Geometry: final body of the model. Coordinates: model frame, mm. A direction names the side the tool comes from. Give positions to 0.01 mm unless a question says otherwise; leave off trailing zeros. Order: outer loops, then holes, each group sorted by start corner. A loop starts at its lowest first (then second) coordinate and runs counter-clockwise, first axis right, second up. Notation, with made-up numbers: (44.5, -37) -> (78.5, -37) arc R34 cw to (78.5, 2) -> close; hole circle Ø11 at (17.25, -7). An arc over 180 degrees is marked (long way). Write item = value, one per line.
```python
from build123d import *

# Parameters (mm, degrees)
BOSS_EXTRUDE1_DEPTH = 12.7


with BuildPart() as part:
    # Sketch1 → Boss-Extrude1 (new, symmetric)
    with BuildSketch(Plane.XY):
        with BuildLine():
            Line((0, 79.375), (19.05, 79.375))
            Line((19.05, 79.375), (19.05, 69.375))
            Line((19.05, 69.375), (0, 69.375))
            ThreePointArc((0, 69.375), (-69.375, 0), (0, -69.375))
            Line((0, -69.375), (19.05, -69.375))
            Line((19.05, -69.375), (19.05, -79.375))
            Line((19.05, -79.375), (0, -79.375))
            ThreePointArc((0, -79.375), (-79.375, 0), (0, 79.375))
        make_face()
    extrude(amount=BOSS_EXTRUDE1_DEPTH, both=True)


solid = part.part
```
1) Section query A-A (z = -8.5). Output: boundary loops of the cut face in (x, y) (3 decimals).
Check sheet entries:
outline = (0, -79.375) -> (19.05, -79.375) -> (19.05, -69.375) -> (0, -69.375) arc R69.375 cw to (0, 69.375) -> (19.05, 69.375) -> (19.05, 79.375) -> (0, 79.375) arc R79.375 ccw to start
2) Section query C-C (y = 52). Output: boundary loops of the cut face in (x, z).
Check sheet entries:
outline = (-59.97, -12.7) -> (-45.92, -12.7) -> (-45.92, 12.7) -> (-59.97, 12.7) -> close
3) Line query: line 1 (Y direction, x = 12.5, z = -7) (3 decimals); line 2 (X direction, y = 1, z = 6.25); line 3 (Y direction, x = -51, z = -8.75). Output: solid intervals per line, ascending. Write a range as from..to.
Check sheet entries:
line_1 = -79.375..-69.375, 69.375..79.375
line_2 = -79.37..-69.37
line_3 = -60.82..-47.03, 47.03..60.82
4) Reachability of faces 5 (the face through (-70, -6, 12.7)), 6 (the face through (10, 69.375, 0)) from +Z, -Z, +X, -X, +Y, -Y: full face, straight path, thin tool, end or side. Return the list, or none.
Check sheet entries:
face_5 = +Z, +X, -X, +Y, -Y
face_6 = +Z, -Z, +X
5) Section query B-B (y = -2.5). Output: boundary loops of the cut face in (x, z).
Check sheet entries:
outline = (-79.34, -12.7) -> (-69.33, -12.7) -> (-69.33, 12.7) -> (-79.34, 12.7) -> close
6) First-contact query: P1, Ø12, axis at x = -31, z = 0, coming from the -Y side; P2, Ø4, axis at y = 49, z = -2.5, coming from the +X side; P3, Ø5, axis at y = -54.5, z = 3.5, coming from the -X side. Flat tips, straight axial feed; report the tip coordinate or a pass-through.
Check sheet entries:
P1 = -75.34
P2 = -47.03
P3 = -59.97
7) Mould query, pull axis Y, two halves, no side actions, for faces 1 (the face through (-70, -6, -12.7)), 2 (the face through (-79.356, -1.745, 0.178)), 3 (the face through (9, 79.375, 0)), 4 (the face through (9, -69.375, 0)). Classes: +Y half, -Y half, draft (parallel to the pull), parting line (faces both ways), or undercut.
Check sheet entries:
face_1 = draft
face_2 = parting line
face_3 = +Y half
face_4 = undercut
